```python
from build123d import *

# Parameters (mm, degrees)
SKETCH1_W                                    = 150
SKETCH1_H                                    = 63
BOSS_EXTRUDE1_DEPTH                          = 8
M4_TAPPED_HOLE1_D                            = 3.3
M4_TAPPED_HOLE1_DEPTH                        = 10.1
M4_TAPPED_HOLE1_TIP                          = 0.991420021
CBORE_FOR_M5_HEXAGON_SOCKET_HEAD_CAP_2_COUNT = 2
CBORE_FOR_M5_HEXAGON_SOCKET_HEAD_CAP_2_PITCH = 28
CBORE_FOR_M5_HEXAGON_SOCKET_HEAD_CAP_3_COUNT = 2
CBORE_FOR_M5_HEXAGON_SOCKET_HEAD_CAP_3_PITCH = 43
CBORE_FOR_M5_HEXAGON_SOCKET_HEAD_CAP_4_COUNT = 2
CBORE_FOR_M5_HEXAGON_SOCKET_HEAD_CAP_4_PITCH = 51.312766443
M2_TAPPED_HOLE1_D                            = 1.6
M2_TAPPED_HOLE1_DEPTH                        = 6.2
M2_TAPPED_HOLE1_TIP                          = 0.480688495
SKETCH17_W                                   = 7
SKETCH17_H                                   = 63
CUT_EXTRUDE1_DEPTH                           = 1
CHAMFER1_SIZE                                = 5


with BuildPart() as part:
    # Sketch1 → Boss-Extrude1 (new body)
    with BuildSketch(Plane(origin=(0, 0, 0), x_dir=(0, 0, -1), z_dir=(1, 0, 0))):
        Rectangle(SKETCH1_W, SKETCH1_H)
    extrude(amount=BOSS_EXTRUDE1_DEPTH)

    # M4 Tapped Hole1
    with Locations(Plane.ZY):
        with Locations((-11, 24), (-11, 5.5)):
            Hole(M4_TAPPED_HOLE1_D / 2, depth=M4_TAPPED_HOLE1_DEPTH)
            with Locations((0, 0, -(M4_TAPPED_HOLE1_DEPTH + M4_TAPPED_HOLE1_TIP / 2))):  # 118° drill point
                Cone(0, M4_TAPPED_HOLE1_D / 2, M4_TAPPED_HOLE1_TIP, mode=Mode.SUBTRACT)

    # Sketch15 → CBORE for M5 Hexagon socket head cap screws1 (revolve, cut)
    with BuildSketch(Plane(origin=(0, 21, 21.5), x_dir=(0, 0, 1), z_dir=(0, 1, 0))):
        Polygon((0, 0), (0, 14.052366702), (2.75, 12.4), (2.75, 5.7), (5, 5.7), (5, 0.025), (5.025, 0), align=None)
    cbore_for_m5_hexagon_socket_head_cap_scr = revolve(axis=Axis((-6.35, 21, 21.5), (1, 0, 0)), mode=Mode.SUBTRACT)

    # CBORE for M5 Hexagon socket head cap 2: CBORE for M5 Hexagon socket head cap screws1 ×2
    with Locations(*[(0, -i * CBORE_FOR_M5_HEXAGON_SOCKET_HEAD_CAP_2_PITCH, 0) for i in range(1, CBORE_FOR_M5_HEXAGON_SOCKET_HEAD_CAP_2_COUNT)]):
        add(cbore_for_m5_hexagon_socket_head_cap_scr, mode=Mode.SUBTRACT)

    # CBORE for M5 Hexagon socket head cap 3: CBORE for M5 Hexagon socket head cap screws1 ×2
    with Locations(*[(0, 0, -i * CBORE_FOR_M5_HEXAGON_SOCKET_HEAD_CAP_3_PITCH) for i in range(1, CBORE_FOR_M5_HEXAGON_SOCKET_HEAD_CAP_3_COUNT)]):
        add(cbore_for_m5_hexagon_socket_head_cap_scr, mode=Mode.SUBTRACT)

    # CBORE for M5 Hexagon socket head cap 4: CBORE for M5 Hexagon socket head cap screws1 ×2
    with Locations(*[Vector(0, -0.5456731714374324, -0.8379980847074858) * (i * CBORE_FOR_M5_HEXAGON_SOCKET_HEAD_CAP_4_PITCH) for i in range(1, CBORE_FOR_M5_HEXAGON_SOCKET_HEAD_CAP_4_COUNT)]):
        add(cbore_for_m5_hexagon_socket_head_cap_scr, mode=Mode.SUBTRACT)

    # M2 Tapped Hole1
    with Locations(Plane.ZY):
        with Locations((-65, 18.5), (-65, 3.5), (-65, -11.5), (65, -11.5), (65, 3.5), (65, 18.5)):
            Hole(M2_TAPPED_HOLE1_D / 2, depth=M2_TAPPED_HOLE1_DEPTH)
            with Locations((0, 0, -(M2_TAPPED_HOLE1_DEPTH + M2_TAPPED_HOLE1_TIP / 2))):  # 118° drill point
                Cone(0, M2_TAPPED_HOLE1_D / 2, M2_TAPPED_HOLE1_TIP, mode=Mode.SUBTRACT)

    # Sketch17 → Cut-Extrude1 (cut)
    with BuildSketch(Plane.ZY):
        with Locations((65, 0)):
            Rectangle(SKETCH17_W, SKETCH17_H)
        with Locations((-65, 0)):
            Rectangle(SKETCH17_W, SKETCH17_H)
    extrude(amount=-CUT_EXTRUDE1_DEPTH, mode=Mode.SUBTRACT)

    # Chamfer1
    chamfer1_edges = [part.edges().sort_by_distance(p)[0] for p in [
        (4, -31.5, -75),
        (4, -31.5, 75),
        (4, 31.5, 75),
        (4, 31.5, -75),
    ]]
    chamfer(chamfer1_edges, length=CHAMFER1_SIZE)


solid = part.part
```
Verification items for the finished model (mm, model axes). A direction names the side the tool comes from. Give positions to 0.01 mm unless a question says otherwise; leave off trailing zeros. Order: outer loops, then holes, each group sorted by start corner. A loop starts at its lowest first (then second) coordinate and runs counter-clockwise, first axis right, second up. Notation, with made-up numbers: (8.5, -40) - (12.5, -40) arc R20 ccw to (12.5, -27) - close; hole circle Ø6 at (-39.75, 51.25). An arc over 180 degrees is marked (long way). Answer as CSV lines item,"result". Start each with the question number.
Item 1: Mould release check, pull along Y, two halves, no side actions. Record for faces 3 (the face through (5.7, -5, -24)), 4 (the face through (3.9, -29, 72.5)), 5 (the face through (8, 0, 1)), 6 (the face through (3.9, 29, -72.5)): released by +Y, released by -Y, zero draft, split by the parting line, or undercut.
Item 2: Section check B-B, the plane x = 4. State how many separate pieces and enclosed holes the cut face has, plus the area to 3 significant figures.
Item 3: Section check A-A, the plane z = -11. Record the boundary of the cut face in (x, y), plus the area to 3 significant figures.
Item 4: Gauge pin test, flat ends, axial feed: pin 1 (3 mm diameter, centred on y = 21, z = 21.5, fed in from -X); pin 2 (6.5 mm diameter, centred on y = -7, z = -21.5, fed in from -X); pin 3 (1.8 mm diameter, centred on y = 3.5, z = 65, fed in from -X). Record the tip position at first contact, or that the pin passes through.
Item 5: Access from +Z, -Z, +X, -X, +Y, -Y to the whole of each face (thin tool, end or side, straight path). Record for faces 1 (the face through (2.82, -8.5, -16.73)), 2 (the face through (0, 0, 1)).
Item 6: Material ranges on L1, parallel to Z at x = 6.7, y = -7; L2, parallel to Z at x = 3.9, y = 21; L3, parallel to Y at x = 4.35, z = 21.5, recorded low to high.
Item 7: Section check D-D, the plane z = 21.5. Record the boundary of the cut face in (x, y) (3 decimals).
Filled in:
1,face 3,"undercut"
1,face 4,"released by -Y"
1,face 5,"zero draft"
1,face 6,"released by +Y"
2,separate pieces,"1"
2,enclosed holes,"12"
2,area,"9,060 mm^2"
3,outline,"(0, -31.5) - (8, -31.5) - (8, 3.85) - (0, 3.85) - close; (0, 7.15) - (8, 7.15) - (8, 22.35) - (0, 22.35) - close; (0, 25.65) - (8, 25.65) - (8, 31.5) - (0, 31.5) - close"
3,area,"451 mm^2"
4,pin 1,"through"
4,pin 2,"x = 5.7"
4,pin 3,"x = 1"
5,face 1,"-X"
5,face 2,"+Z, -Z, -X, +Y, -Y"
6,L1,"-75 to -24.25, -18.75 to 18.75, 24.25 to 75"
6,L2,"-75 to -26.5, -16.5 to 16.5, 26.5 to 75"
6,L3,"-31.5 to -12, -2 to 16, 26 to 31.5"
7,outline,"(0, -31.5) - (8, -31.5) - (8, -9.75) - (5.7, -9.75) - (5.7, -12) - (0.025, -12) - (0, -12.025) - close; (0, -1.975) - (0.025, -2) - (5.7, -2) - (5.7, -4.25) - (8, -4.25) - (8, 18.25) - (5.7, 18.25) - (5.7, 16) - (0.025, 16) - (0, 15.975) - close; (0, 26.025) - (0.025, 26) - (5.7, 26) - (5.7, 23.75) - (8, 23.75) - (8, 31.5) - (0, 31.5) - close"
